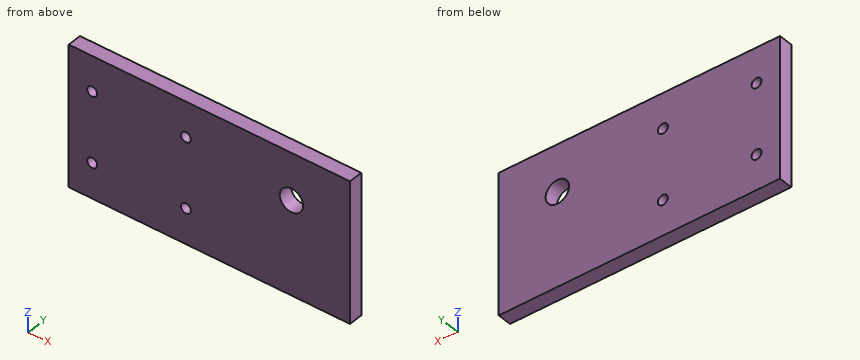
```python
from build123d import *

# Parameters (mm, degrees)
SKETCH_1_W      = 240
SKETCH_1_H      = 120
SKETCH_1_R      = 4.25
SKETCH_1_R_2    = 10
EXTRUDE_1_DEPTH = 12


with BuildPart() as part:
    # 草图1 → 凸台-拉伸1 (new body)
    with BuildSketch(Plane(origin=(0, 0, 0), x_dir=(1, 0, 0), z_dir=(0, 1, 0))):
        with Locations((120, 60)):
            Rectangle(SKETCH_1_W, SKETCH_1_H)
        with Locations(Location((20, 30, 0), (0, 0, 270))):
            Circle(SKETCH_1_R, mode=Mode.SUBTRACT)
        with Locations(Location((20, 90, 0), (0, 0, 270))):
            Circle(SKETCH_1_R, mode=Mode.SUBTRACT)
        with Locations(Location((100, 90, 0), (0, 0, 270))):
            Circle(SKETCH_1_R, mode=Mode.SUBTRACT)
        with Locations(Location((100, 30, 0), (0, 0, 270))):
            Circle(SKETCH_1_R, mode=Mode.SUBTRACT)
        with Locations(Location((190, 40, 0), (0, 0, 270))):
            Circle(SKETCH_1_R_2, mode=Mode.SUBTRACT)
    extrude(amount=EXTRUDE_1_DEPTH)


solid = part.part
```
Geometry check sheet. Reference: the model listing, model coordinates, mm. Coordinates: 2 decimals unless noted, no trailing zeros. Order: outer loops, then holes, each group sorted by start corner. A loop starts at its lowest first (then second) coordinate and runs counter-clockwise, first axis right, second up. Notation, with made-up numbers: (7.5, 56.5) - (41.5, 56.5) arc R19 cw to (41.5, 77.5) - close; hole circle Ø8 at (21, 24.25). An arc over 180 degrees is marked (long way). Answer as a JSON object with one key per item and string values. Group by question number.
Item 1: Sectioned sample at A-A, the plane z = -40. Record the cut outline in (x, y).
Item 2: Sectioned sample at B-B, the plane x = 20. Record the cut outline in (y, z).
Item 3: Sectioned sample at C-C, the plane y = 3.5. Record the cut outline in (x, z), and give its area (3 significant figures).
Item 4: Depth check by flat-ended pin: pin 1 Ø13.5 at (x, z) = (100, -30) entering from +Y; pin 2 Ø7.5 at (x, z) = (20, -90) entering from +Y. Enter the tip coordinate at first touch or a pass-through.
Item 5: Scan lines: probe 1 along X at (y, z) = (3, -90); probe 2 along X at (y, z) = (6.5, -40); probe 3 along Z at (x, y) = (99, 5.25). Record each from-to range of solid material in increasing order.
Resolved:
{
 "1": {"outline": "(0, 0) - (180, 0) - (180, 12) - (0, 12) - close; (200, 0) - (240, 0) - (240, 12) - (200, 12) - close"},
 "2": {"outline": "(0, -120) - (12, -120) - (12, -94.25) - (0, -94.25) - close; (0, -85.75) - (12, -85.75) - (12, -34.25) - (0, -34.25) - close; (0, -25.75) - (12, -25.75) - (12, 0) - (0, 0) - close"},
 "3": {"outline": "(0, -120) - (240, -120) - (240, 0) - (0, 0) - close; hole circle Ø8.5 at (20, -90); hole circle Ø8.5 at (20, -30); hole circle Ø8.5 at (100, -90); hole circle Ø8.5 at (100, -30); hole circle Ø20 at (190, -40)", "area": "28,300 mm^2"},
 "4": {"pin 1": "y = 12", "pin 2": "through"},
 "5": {"probe 1": "0 to 15.75, 24.25 to 95.75, 104.25 to 240", "probe 2": "0 to 180, 200 to 240", "probe 3": "-120 to -94.13, -85.87 to -34.13, -25.87 to 0"}
}
